from build123d import *

# Parameters (mm, degrees)
SKETCH1_R           = 10
SKETCH1_R_2         = 5
BOSS_EXTRUDE1_DEPTH = 4


with BuildPart() as part:
    # Sketch1 → Boss-Extrude1 (new, symmetric)
    with BuildSketch(Plane.XY):
        Polygon((0, 0), (0, 180), (40, 180), (40, 10), align=None)
        with Locations((20, 160)):
            Circle(SKETCH1_R, mode=Mode.SUBTRACT)
        with Locations((32, 90)):
            Circle(SKETCH1_R_2, mode=Mode.SUBTRACT)
        with Locations((32, 55)):
            Circle(SKETCH1_R_2, mode=Mode.SUBTRACT)
        with Locations((32, 20)):
            Circle(SKETCH1_R_2, mode=Mode.SUBTRACT)
    extrude(amount=BOSS_EXTRUDE1_DEPTH, both=True)


solid = part.part
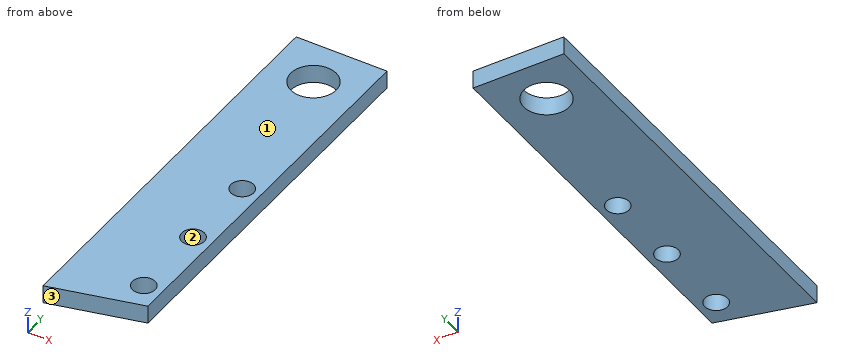
Geometry: final body of the model. Coordinates: model frame, mm. Face numbers are marked on the shaded views. Round coordinates to 2 decimals unless told otherwise and drop trailing zeros. Loops run counter-clockwise (first coordinate to the right, second up) from the corner with the lowest first, then second, coordinate; pieces in that order, holes last. Notation, with made-up numbers: (80.5, 74) -> (133.5, 74) arc R5 ccw to (133.5, 83) -> close; hole circle Ø3 at (26, -38). An arc over 180 degrees is marked (long way). One line per question, with ' | ' between items. Start each with the question number.
1. Line query: line 1 along Y through (x, z) = (32, -2); line 2 along Y through (x, z) = (12.5, -2.75) (3 decimals); line 3 along X through (y, z) = (163.5, 2.75). Output: solid intervals per line, ascending. Write a range as [from, to].
2. Section B-B on z = 2.75. Output: boundary loops of the cut face in (x, y), and give its area (3 significant figures).
3. Section A-A on x = 20. Output: boundary loops of the cut face in (y, z), and give its area (3 significant figures).
4. Section D-D on x = 32. Output: boundary loops of the cut face in (y, z), and give its area (3 significant figures).
5. Contact query for flat-ended pins moving along their axis: pin 1 (1 mm diameter, centred on x = 26.5, z = 2, fed in from -Y); pin 2 (16 mm diameter, centred on x = 20, y = 160, fed in from +Z). Output: stop coordinate, or through.
6. Mould query, pull axis Y, two halves, no side actions, for the marked faces 1, 2 and 3. Classes: pulls with the +Y half, pulls with the -Y half, needs draft (parallel to the pull), parting line crosses it, or undercut.
7. Section C-C on y = 160. Output: boundary loops of the cut face in (x, z).
Returned:
1) line 1: y = [8, 15], [25, 50], [60, 85], [95, 180] | line 2: y = [3.125, 153.386], [166.614, 180] | line 3: x = [0, 10.63], [29.37, 40]
2) outline: (0, 0) -> (40, 10) -> (40, 180) -> (0, 180) -> close; hole circle Ø20 at (20, 160); hole circle Ø10 at (32, 20); hole circle Ø10 at (32, 55); hole circle Ø10 at (32, 90) | area: 6,450 mm2
3) outline: (5, -4) -> (150, -4) -> (150, 4) -> (5, 4) -> close; (170, -4) -> (180, -4) -> (180, 4) -> (170, 4) -> close | area: 1,240 mm2
4) outline: (8, -4) -> (15, -4) -> (15, 4) -> (8, 4) -> close; (25, -4) -> (50, -4) -> (50, 4) -> (25, 4) -> close; (60, -4) -> (85, -4) -> (85, 4) -> (60, 4) -> close; (95, -4) -> (180, -4) -> (180, 4) -> (95, 4) -> close | area: 1,140 mm2
5) pin 1: stops at y = 6.5 | pin 2: passes through
6) face 1: needs draft | face 2: undercut | face 3: pulls with the -Y half
7) outline: (0, -4) -> (10, -4) -> (10, 4) -> (0, 4) -> close; (30, -4) -> (40, -4) -> (40, 4) -> (30, 4) -> close
